Verification items for the finished model (mm, model axes). A direction names the side the tool comes from. Coordinates: 2 decimals unless noted, no trailing zeros. Order: outer loops, then holes, each group sorted by start corner. A loop starts at its lowest first (then second) coordinate and runs counter-clockwise, first axis right, second up. Notation, with made-up numbers: (25, -11) -> (54, -11) arc R6 ccw to (54, -2) -> close; hole circle Ø2 at (56, 75). An arc over 180 degrees is marked (long way). Write each question's results on one line, items separated by ' | '. Start each with the question number.
(1) Go/stop test with flat-tipped pins: pin 1 (4 mm diameter, centred on y = -7, z = 78.5, fed in from +X); pin 2 (2.5 mm diameter, centred on y = -2, z = 71.5, fed in from +X); pin 3 (8 mm diameter, centred on x = 91, z = 55, fed in from -Y); pin 4 (3 mm diameter, centred on y = -5, z = 50, fed in from +X). Record where each tip stops, or that it passes through.
(2) Cross-section at B-B on x = 28. Enter the section's corners in (y, z), and give its area (3 significant figures).
(3) Thickness scan on probe 1 along Z at (x, y) = (-187.5, -44.5); probe 2 along Z at (x, y) = (259, -44) (3 decimals); probe 3 along Y at (x, z) = (269, 17.5). Record the ranges inside material, lowest first. Write a range as [from, to].
(4) Draft check along Z on faces 3 (the flat face through (5.6, -28.782, 8.287)), 4 (the flat face through (6, -24, 0)), 5 (the flat face through (-400, -18, 6)), 6 (the flat face through (5.6, -28.35, 91.67)). Enter one of: +Z half, -Z half, draft (parallel to the pull), parting line (faces both ways), or undercut.
(5) Cross-section at A-A on x = 140.5. Enter the section's corners in (y, z).
(6) Cross-section at D-D on z = 50. Enter the section's corners in (x, y), and give its area (3 significant figures).
(7) Cross-section at C-C on y = -22.5. Enter the section's corners in (x, z) (3 decimals), and give its area (3 significant figures).
(8) Set-up check for faces 1 (the flat face through (6, 0, 51)), 2 (the flat face through (6, -5.3, 50)): record each of +Z, -Z, +X, -X, +Y, -Y from which the full face is reachable in a straight line by a thin tool's end or side.
```python
from build123d import *

# Parameters (mm, degrees)
HOT_ROLLED_CHANNEL_STEEL_GB_T_707_1988_DEPTH = 800
CUT_EXTRUDE1_DEPTH                           = 10
SKETCH4_W                                    = 25
SKETCH4_H                                    = 15
CUT_EXTRUDE2_DEPTH                           = 10


with BuildPart() as part:
    # Sketch1 → hot-rolled channel steel (GB/T 707-1988) 10(1) (new body)
    with BuildSketch(Plane(origin=(400, 0, 0), x_dir=(0, -1, 0), z_dir=(-1, 0, 0))):
        with BuildLine():
            Line((48, 100), (0, 100))
            Line((0, 100), (0, 0))
            Line((0, 0), (48, 0))
            Line((48, 0), (48, 2.518802861))
            ThreePointArc((48, 2.518802861), (46.901173268, 5.370575474), (44.172890806, 6.747710919))
            Line((44.172890806, 6.747710919), (12.954218388, 9.869578161))
            ThreePointArc((12.954218388, 9.869578161), (7.497653465, 12.623849051), (5.3, 18.327394278))
            Line((5.3, 18.327394278), (5.3, 81.672605722))
            ThreePointArc((5.3, 81.672605722), (7.497653465, 87.376150949), (12.954218388, 90.130421839))
            Line((12.954218388, 90.130421839), (44.172890806, 93.252289081))
            ThreePointArc((44.172890806, 93.252289081), (46.901173268, 94.629424526), (48, 97.481197139))
            Line((48, 97.481197139), (48, 100))
        make_face()
    extrude(amount=HOT_ROLLED_CHANNEL_STEEL_GB_T_707_1988_DEPTH)

    # Sketch3 → Cut-Extrude1 (cut)
    with BuildSketch(Plane(origin=(0, 0, 0), x_dir=(1, 0, 0), z_dir=(0, 1, 0))):
        with BuildLine():
            Line((-680, -37), (-120, -37))
            ThreePointArc((-120, -37), (-107, -50), (-120, -63))
            Line((-120, -63), (-680, -63))
            ThreePointArc((-680, -63), (-693, -50), (-680, -37))
        make_face()
    cut_extrude1 = extrude(amount=-CUT_EXTRUDE1_DEPTH, mode=Mode.SUBTRACT)

    # Sketch4 → Cut-Extrude2 (cut)
    with BuildSketch(Plane(origin=(0, 0, 0), x_dir=(1, 0, 0), z_dir=(0, 1, 0))):
        with Locations((-387.5, -29.5)):
            Rectangle(SKETCH4_W, SKETCH4_H)
        with Locations((-387.5, -70.5)):
            Rectangle(SKETCH4_W, SKETCH4_H)
    cut_extrude2 = extrude(amount=-CUT_EXTRUDE2_DEPTH, mode=Mode.SUBTRACT)

    # Mirror1: Cut-Extrude1, Cut-Extrude2 across plane
    add(cut_extrude1.mirror(Plane(origin=(0, 0, 0), x_dir=(0, 0, 1), z_dir=(1, 0, 0))), mode=Mode.SUBTRACT)
    add(cut_extrude2.mirror(Plane(origin=(0, 0, 0), x_dir=(0, 0, 1), z_dir=(1, 0, 0))), mode=Mode.SUBTRACT)


solid = part.part
```
Results are:
1) pin 1: stops at x = 400 | pin 2: stops at x = 375 | pin 3: stops at y = -5.3 | pin 4: stops at x = 107.09
2) outline: (-48, 0) -> (0, 0) -> (0, 100) -> (-48, 100) -> (-48, 97.48) arc R4.25 ccw to (-44.17, 93.25) -> (-12.95, 90.13) arc R8.5 cw to (-5.3, 81.67) -> (-5.3, 18.33) arc R8.5 cw to (-12.95, 9.87) -> (-44.17, 6.75) arc R4.25 ccw to (-48, 2.52) -> close | area: 1,270 mm2
3) probe 1: z = [0, 6.7], [93.3, 100] | probe 2: z = [0, 6.765], [93.235, 100] | probe 3: y = [-5.34, 0]
4) face 3: undercut | face 4: -Z half | face 5: draft | face 6: undercut
5) outline: (-48, 0) -> (0, 0) -> (0, 37) -> (-5.3, 37) -> (-5.3, 18.33) arc R8.5 cw to (-12.95, 9.87) -> (-44.17, 6.75) arc R4.25 ccw to (-48, 2.52) -> close; (-48, 97.48) arc R4.25 ccw to (-44.17, 93.25) -> (-12.95, 90.13) arc R8.5 cw to (-5.3, 81.67) -> (-5.3, 63) -> (0, 63) -> (0, 100) -> (-48, 100) -> close
6) outline: (-107, -5.3) -> (107, -5.3) -> (107, 0) -> (-107, 0) -> close | area: 1,130 mm2
7) outline: (-400, 0) -> (400, 0) -> (400, 8.915) -> (-400, 8.915) -> close; (-400, 91.085) -> (400, 91.085) -> (400, 100) -> (-400, 100) -> close | area: 14,300 mm2
8) face 1: +Z, -Z, +X, -X, +Y | face 2: +X, -X, -Y
